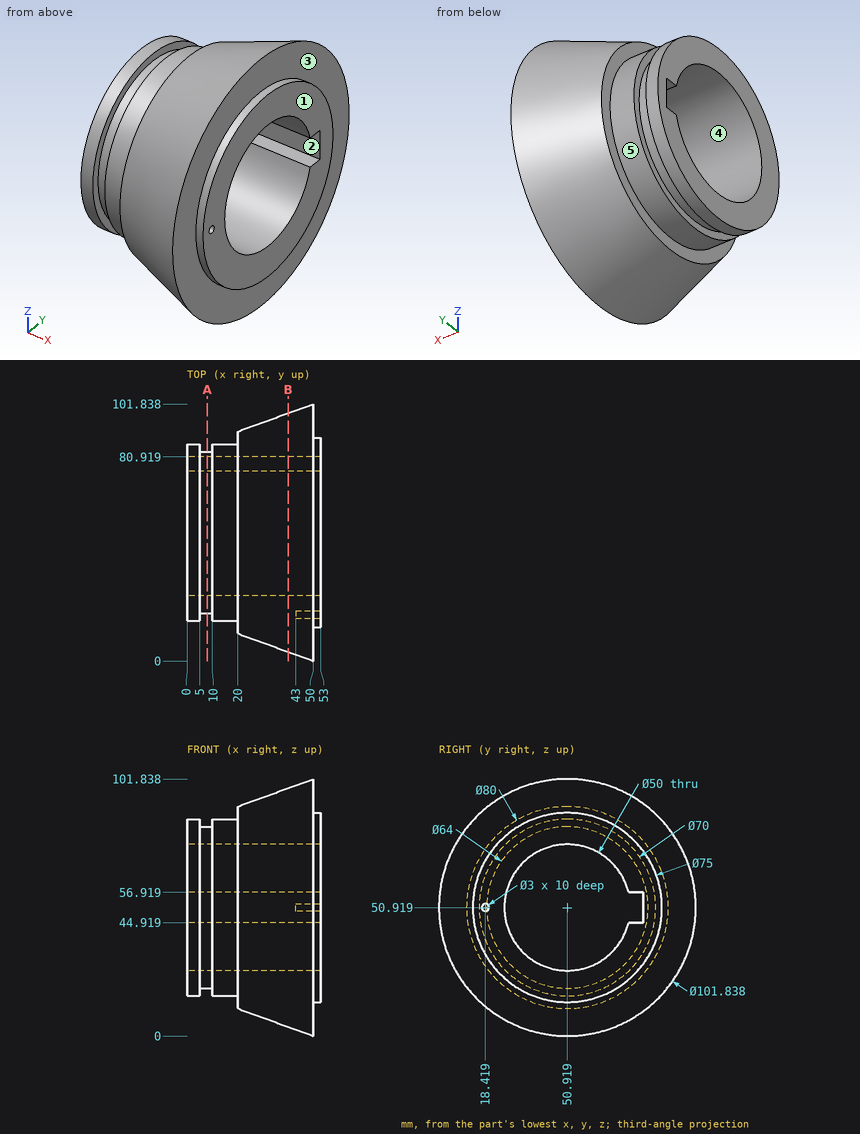
Geometry: see drawing. Coordinates: mm, zero at the bounding-box minimum. A direction names the side the tool comes from. Round coordinates to 2 decimals unless told otherwise and drop trailing zeros. Order: outer loops, then holes, each group sorted by start corner. A loop starts at its lowest first (then second) coordinate and runs counter-clockwise, first axis right, second up. Notation, with made-up numbers: (72, -33.5) - (113, -33.5) arc R35 ccw to (113, 2.5) - close; hole circle Ø6 at (-11, 51). An arc over 180 degrees is marked (long way). Use a Markdown table: item, result. Add a question column.
1. Set-up query: the marked faces 1 and 2. Return all of +Z, -Z, +X, -X, +Y, -Y with unobstructed straight access to the full face (end or side cutting, diameter ignored); none if empty.
2. Line query: probe 1 along Z at (x, y) = (15, 60.5); probe 2 along X at (y, z) = (55.5, 12); probe 3 along Y at (x, z) = (9, 35.5). Output: solid intervals per line, ascending.
3. Section query A-A (x = 8). Return the cut outline in (y, z), then the cut area to 3 significant figures.
4. Section query B-B (x = 40). Return the cut outline in (y, z), then the cut area to 3 significant figures.
5. Mould query, pull axis Y, two halves, no side actions, for the marked faces 3, 4 and 5. Classes: +Y half, -Y half, draft (parallel to the pull), parting line (faces both ways), or undercut.
6. First-contact query: pin 1 (1.8 mm diameter, centred on y = 18.42, z = 50.92, fed in from +X); pin 2 (4 mm diameter, centred on y = 89.5, z = 21.5, fed in from +X); pin 3 (3 mm diameter, centred on x = 19, y = 77, fed in from +Z). Flat tips, straight axial feed; report the tip coordinate or a pass-through.
Derived:
| question | item | result |
|---|---|---|
| 1 | face 1 | +Z, -Z, +X, +Y, -Y |
| 1 | face 2 | +X, -X |
| 2 | probe 1 | 17.26 to 27.83, 74.01 to 84.58 |
| 2 | probe 2 | 20 to 50 |
| 2 | probe 3 | 22.88 to 31.24, 70.6 to 78.96 |
| 3 | outline | circle Ø64 at (50.92, 50.92); hole (75.19, 44.92) - (80.92, 44.92) - (80.92, 56.92) - (75.19, 56.92) arc R25 ccw (long way) to start |
| 3 | area | 1,190 mm2 |
| 4 | outline | circle Ø94.56 at (50.92, 50.92); hole (75.19, 44.92) - (80.92, 44.92) - (80.92, 56.92) - (75.19, 56.92) arc R25 ccw (long way) to start |
| 4 | area | 5,000 mm2 |
| 5 | face 3 | draft |
| 5 | face 4 | undercut |
| 5 | face 5 | parting line |
| 6 | pin 1 | x = 43 |
| 6 | pin 2 | x = 50 |
| 6 | pin 3 | z = 82.17 |
